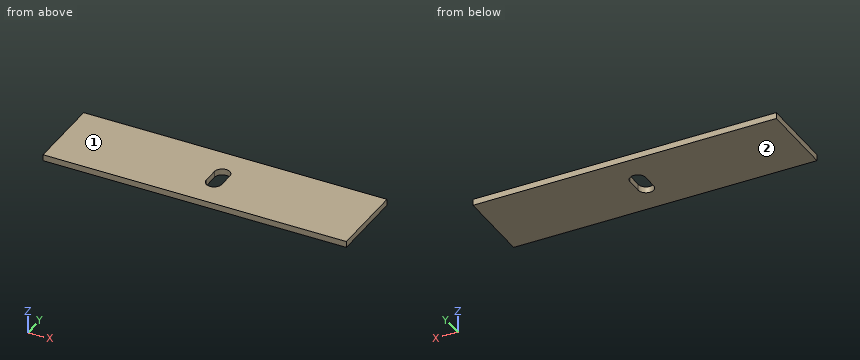
from build123d import *

# Parameters (mm, degrees)
BOSS_EXTRUDE1_DEPTH = 20


with BuildPart() as part:
    # Sketch1 → Boss-Extrude1 (new body)
    with BuildSketch(Plane.XY):
        Polygon((11341.12511676, 4637.824188368), (11341.125116846, 4387.824188368), (12321.125115149, 4387.824188368), (12321.125115149, 4637.824188368), align=None)
        with BuildLine():
            Line((11816.125116094, 4537.824187896), (11816.125116094, 4487.824187992))
            ThreePointArc((11816.125116094, 4487.824187992), (11841.125216971, 4462.824188038), (11866.125116001, 4487.824389839))
            Line((11866.125116001, 4487.824389839), (11866.125116001, 4537.823600328))
            ThreePointArc((11866.125116001, 4537.823600328), (11841.125409832, 4562.823894066), (11816.125116094, 4537.824187896))
        make_face(mode=Mode.SUBTRACT)
    extrude(amount=BOSS_EXTRUDE1_DEPTH)


solid = part.part
Here's how the part is built. I have some questions about the finished solid (model axes, mm). Face numbers are marked on the shaded views. Round coordinates to 2 decimals unless told otherwise and drop trailing zeros. Order: outer loops, then holes, each group sorted by start corner. A loop starts at its lowest first (then second) coordinate and runs counter-clockwise, first axis right, second up. Notation, with made-up numbers: M 88.5,-6.5 L 139.5,-6.5 A15 ccw 139.5,8.5 Z; hole C 7,55.25 d8. An arc over 180 degrees is marked long. Return JSON: item names as keys, results as strings. Group by question number.
1. If we section it at C-C on x = 11857: List the corners of the cut face in (y, z) for me.
2. I'm going to push a flat-ended pin straight in: pin 1 Ø10 at (x, y) = (11993, 4482) entering from -Z. Where does the tip first touch, or does it pass through?
3. If we section it at B-B on z = 7.5: List the corners of the cut face in (x, y) for me.
4. If we mould it in two halves opening along Z, with no side actions, what happens to the marked faces 1 and 2? For each: pulls with the +Z half, pulls with the -Z half, needs draft (parallel to the pull), parting line crosses it, or undercut.
5. Please list where these lines run through material, in increasing order: probe 1 along X at (y, z) = (4512, 10.5); probe 2 along X at (y, z) = (4539.5, 6.75).
6. If we section it at A-A on y = 4519: List the corners of the cut face in (x, z) for me.
Reply:
{
 "1": {"outline": "M 4387.82,0 L 4468.51,0 L 4468.51,20 L 4387.82,20 Z; M 4557.14,0 L 4637.82,0 L 4637.82,20 L 4557.14,20 Z"},
 "2": {"pin 1": "z = 0"},
 "3": {"outline": "M 11341.13,4387.82 L 12321.13,4387.82 L 12321.13,4637.82 L 11341.13,4637.82 Z; hole M 11816.13,4487.82 A25 ccw 11866.13,4487.82 L 11866.13,4537.82 A25 ccw 11816.13,4537.82 Z"},
 "4": {"face 1": "pulls with the +Z half", "face 2": "pulls with the -Z half"},
 "5": {"probe 1": "11341.13 to 11816.13, 11866.13 to 12321.13", "probe 2": "11341.13 to 11816.18, 11866.07 to 12321.13"},
 "6": {"outline": "M 11341.13,0 L 11816.13,0 L 11816.13,20 L 11341.13,20 Z; M 11866.13,0 L 12321.13,0 L 12321.13,20 L 11866.13,20 Z"}
}
